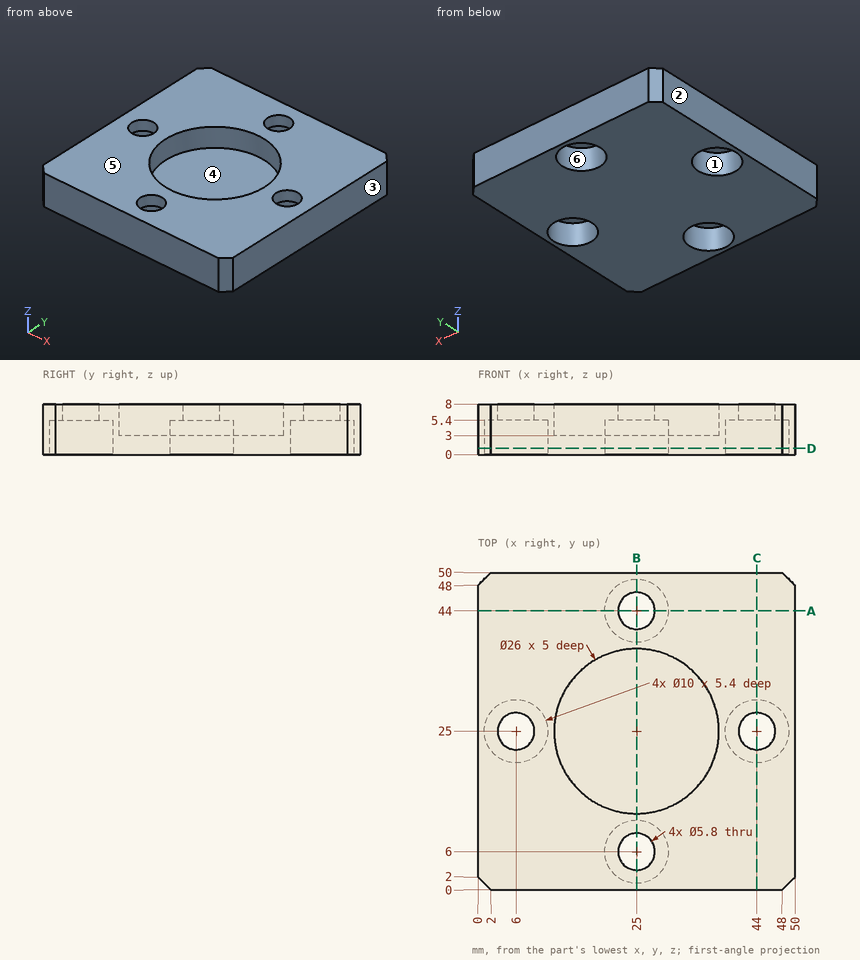
Check sheet for the drawn part. Datum: minimum x, y, z corner. Units: mm. A direction names the side the tool comes from. Give positions to 0.01 mm unless a question says otherwise; leave off trailing zeros. Write each loop counter-clockwise with the first axis right and the second up, starting at its lowest first coordinate (ties: lowest second). Pieces come first, ordered by that corner, then holes. Notation, with made-up numbers: (-37.75, 76.5) -> (-17.75, 76.5) arc R27 ccw to (-17.75, 115.5) -> close; hole circle Ø4 at (83, -9). An arc over 180 degrees is marked (long way). Use one line per item in the form item = value. Start each with the question number.
1. Thickness scan on line 1 along Y through (x, z) = (25, 2.2); line 2 along Y through (x, z) = (25, 6.05); line 3 along Y through (x, z) = (25, 5.2). Record the ranges inside material, lowest first. Write a range as from..to.
2. Section check B-B (x = 25). Record the cut outline in (y, z).
3. Section check A-A (y = 44). Record the cut outline in (x, z), and give its area (3 significant figures).
4. Mould release check, pull along X, two halves, no side actions. Record for the marked faces 1, 2 and 3: pulls with the +X half, pulls with the -X half, needs draft (parallel to the pull), parting line crosses it, or undercut.
5. Access from +Z, -Z, +X, -X, +Y, -Y to the whole of each face (thin tool, end or side, straight path). Record for the marked faces 4, 5 and 6.
6. Go/stop test with flat-tipped pins: P1, Ø6.5, axis at x = 25, y = 6, coming from the -Z side; P2, Ø3.5, axis at x = 44, y = 25, coming from the +Z side. Record where each tip stops, or that it passes through.
7. Section check D-D (z = 1). Record the cut outline in (x, y), and give its area (3 significant figures).
Conclusion:
q1.line_1 = 0..1, 11..39, 49..50
q1.line_2 = 0..3.1, 8.9..12, 38..41.1, 46.9..50
q1.line_3 = 0..1, 11..12, 38..39, 49..50
q2.outline = (0, 0) -> (1, 0) -> (1, 5.4) -> (3.1, 5.4) -> (3.1, 8) -> (0, 8) -> close; (8.9, 5.4) -> (11, 5.4) -> (11, 0) -> (39, 0) -> (39, 5.4) -> (41.1, 5.4) -> (41.1, 8) -> (38, 8) -> (38, 3) -> (12, 3) -> (12, 8) -> (8.9, 8) -> close; (46.9, 5.4) -> (49, 5.4) -> (49, 0) -> (50, 0) -> (50, 8) -> (46.9, 8) -> close
q3.outline = (0, 0) -> (20, 0) -> (20, 5.4) -> (22.1, 5.4) -> (22.1, 8) -> (0, 8) -> close; (27.9, 5.4) -> (30, 5.4) -> (30, 0) -> (50, 0) -> (50, 8) -> (27.9, 8) -> close
q3.area = 331 mm²
q4.face_1 = undercut
q4.face_2 = pulls with the -X half
q4.face_3 = pulls with the +X half
q5.face_4 = +Z
q5.face_5 = +Z, +X, -X, +Y, -Y
q5.face_6 = -Z
q6.P1 = 5.4
q6.P2 = through
q7.outline = (0, 2) -> (2, 0) -> (48, 0) -> (50, 2) -> (50, 48) -> (48, 50) -> (2, 50) -> (0, 48) -> close; hole circle Ø10 at (6, 25); hole circle Ø10 at (25, 6); hole circle Ø10 at (25, 44); hole circle Ø10 at (44, 25)
q7.area = 2,180 mm²
